The model under review builds one solid part; all positions refer to its coordinate system, in mm. A direction names the side the tool comes from. Coordinates: 2 decimals unless noted, no trailing zeros. Order: outer loops, then holes, each group sorted by start corner. A loop starts at its lowest first (then second) coordinate and runs counter-clockwise, first axis right, second up. Notation, with made-up numbers: M 89,76.25 L 102,76.25 A15 ccw 102,99.25 Z; hole C 15.5,40 d7. An arc over 180 degrees is marked long. Answer as CSV lines item,"result". Start each with the question number.
Q1. For P1, Ø9, axis at x = -4, y = 87, coming from the +Z side; P2, Ø3, axis at y = -1, z = -2.5, coming from the -X side; P3, Ø12, axis at x = 21, z = 29, coming from the +Y side, all flat-tipped, find the tip position at first contact; note any pin that passes through.
Q2. Machinability: for faces 1 (the face through (7.4, 25.341, 7.3)), 2 (the face through (8.84, 24.63, -15.52)), 3 (the face through (-9, 25, -15)), 4 (the face through (0, 131, 10)), which of the approach directions +Z, -Z, +X, -X, +Y, -Y give a long, thin tool a straight path to every point of the face, cutting with its end or side? Answer none if there is none.
Q3. Wall thickness on L1, parallel to Y at x = 17, z = -14.5; L2, parallel to Z at x = 14, y = 85.5; L3, parallel to Y at x = -38.5, z = 13: over which ranges is each line inside the solid? List them lowest first. Write a range as [from, to].
Q4. Consider section B-B on y = 155.5. Write out the cut boundary in (x, z).
Q5. The part is to be moulded in two halves that separate along Y. For faces 5 (the face through (17.86, 24.63, -0.1)), 6 (the face through (17.83, 8.02, -0.1)), 7 (the face through (-17.86, 94.63, 0.1)), 8 (the face through (14.8, 16.5, -8.4)), say which applies: +Y half, -Y half, draft (parallel to the pull), parting line (faces both ways), or undercut.
from build123d import *

# Parameters (mm, degrees)
SKETCH_2_R          = 28.577779899
EXTRUDE_1_DEPTH     = 6
SKETCH_4_R          = 24.484212217
CUT_EXTRUDE_5_DEPTH = 88
CHAMFER_1_SIZE      = 1


with BuildPart() as part:
    # 草图1 → 旋转1 (revolve)
    with BuildSketch(Plane.XY, mode=Mode.PRIVATE) as revolve_1_sk:
        Polygon((10, 169.340745793), (10, 95.340745793), (19.65, 95.340745793), (19.65, 77.340745793), (10, 77.340745793), (10, 25.340745793), (19.65, 25.340745793), (19.65, 7.340745793), (10, 7.340745793), (10, 0.340745793), (28.577779899, 0.340745793), (50, -14.659254207), (50, -24.659254207), (0, -24.659254207), (0, 169.340745793), align=None)
    revolve(revolve_1_sk.sketch.rotate(Axis((0, -29.818093999, 0), (0, 1, 0)), 90), axis=Axis((0, -29.818093999, 0), (0, 1, 0)))

    # 草图2 → 凸台-拉伸1 (add)
    with BuildSketch(Plane(origin=(0, 0.340745793, 0), x_dir=(1, 0, 0), z_dir=(0, 1, 0))):
        with Locations(Location((0, 0, 0), (0, 0, 270))):
            Circle(SKETCH_2_R)
    extrude(amount=EXTRUDE_1_DEPTH)

    # 草图4 → 切除-拉伸5 (cut)
    with BuildSketch(Plane(origin=(0, 95.340745793, 0), x_dir=(1, 0, 0), z_dir=(0, 1, 0))):
        Circle(SKETCH_4_R)
        Polygon((19.65, 0), (9.825, 17.017399184), (-9.825, 17.017399184), (-19.65, 0), (-9.825, -17.017399184), (9.825, -17.017399184), align=None, mode=Mode.SUBTRACT)
    extrude(amount=-CUT_EXTRUDE_5_DEPTH, mode=Mode.SUBTRACT)

    # 草图5 → 切除-旋转1 (revolve, cut)
    with BuildSketch(Plane.XY):
        Polygon((-17.15, 95.340745793), (-19.65, 92.840745793), (-26.926915052, 99.124494225), (-16.245783772, 99.906767383), align=None)
        Polygon((-17.15, 77.340745793), (-19.65, 79.840745793), (-19.65, 76.234905644), align=None)
        Polygon((-17.15, 25.340745793), (-19.65, 22.840745793), (-41.601041536, 16.623626451), (-25.840347108, 26.762569484), align=None)
        Polygon((-19.65, 9.840745793), (-17.15, 7.340745793), (-28.367472728, 7.340745793), align=None)
    revolve(axis=Axis((0, 180.885465797, 0), (0, -1, 0)), mode=Mode.SUBTRACT)

    # 倒角1
    chamfer_1_edges = [part.edges().sort_by_distance(p)[0] for p in [
        (0, 169.340745793, 10),
    ]]
    chamfer(chamfer_1_edges, length=CHAMFER_1_SIZE)


solid = part.part
Evaluation:
1,P1,"stops at z = 17.02"
1,P2,"stops at x = -32.54"
1,P3,"stops at y = -0.52"
2,face 1,"none"
2,face 2,"-Z, +X"
2,face 3,"-Z, -X"
2,face 4,"+Y"
3,L1,"y = [-24.66, 6.34]"
3,L2,"z = [-9.79, 9.79]"
3,L3,"y = [-24.66, -8.1]"
4,outline,"C 0,0 d20"
5,face 5,"undercut"
5,face 6,"undercut"
5,face 7,"+Y half"
5,face 8,"draft"
